The model under review builds one solid part; all positions refer to its coordinate system, in mm. Give positions to 0.01 mm unless a question says otherwise; leave off trailing zeros. Order: outer loops, then holes, each group sorted by start corner. A loop starts at its lowest first (then second) coordinate and runs counter-clockwise, first axis right, second up. Notation, with made-up numbers: M 70,16.5 L 87,16.5 A23 cw 87,49.5 Z; hole C -30.5,89 d3. An arc over 180 degrees is marked long. One line per question, with ' | ' between items. Start each with the question number.
1. Wall thickness on L1, parallel to X at y = 83.5, z = 4.25; L2, parallel to Y at x = -50.5, z = 9.5; L3, parallel to Y at x = -45, z = 12.5: over which ranges is each line inside the solid? List them lowest first.
2. We need section D-D on y = 108.5. Write out the cut boundary in (x, z).
3. We need section A-A on y = 63.5. Write out the cut boundary in (x, z).
4. Insertion check: P1, Ø1, axis at x = -27, y = 61.5, coming from the -Z side; P2, Ø10, axis at x = -10, z = 8, coming from the +Y side; P3, Ø10, axis at y = 93.5, z = 5, coming from the +X side; P4, Ø24, axis at x = -45, y = 81, coming from the -Z side. Each pin has a flat end and moves straight along its axis. Give the tip position at first contact, or say it passes through.
5. We need section B-B on x = -30. Write out the cut boundary in (y, z).
6. The part is to be moulded in two halves that separate along X. For faces 1 (the face through (-54.229, 63.257, 9.86)), 2 (the face through (-46, 50, 20)), 3 (the face through (-45.63, 6.785, 9.86)), say which applies: +X half, -X half, draft (parallel to the pull), parting line (faces both ways), or undercut.
7. We need section C-C on z = 4. Write out the cut boundary in (x, y).
```python
from build123d import *

# Parameters (mm, degrees)
EXTRUDE_1_DEPTH     = 20
SKETCH_2_R          = 20
CUT_EXTRUDE_1_DEPTH = 157.12815249


with BuildPart() as part:
    # 草图1 → 凸台-拉伸1 (new body)
    with BuildSketch(Plane.XY):
        with BuildLine():
            Line((0, 0), (0, 81))
            ThreePointArc((0, 81), (-45, 126), (-90, 81))
            Line((-90, 81), (-90, 13.383545734))
            Line((-90, 13.383545734), (0, 0))
        make_face()
    extrude(amount=EXTRUDE_1_DEPTH)

    # 草图2 → 切除-拉伸1 (cut, through all)
    with BuildSketch(Plane(origin=(0, 0, 0), x_dir=(-1, 0, 0), z_dir=(0, 0, -1))):
        with Locations((45, 81)):
            Circle(SKETCH_2_R)
    extrude(amount=-CUT_EXTRUDE_1_DEPTH, mode=Mode.SUBTRACT)


solid = part.part
```
Entries:
1) L1: x = -89.93 to -64.84, -25.16 to -0.07 | L2: y = 7.51 to 61.77, 100.23 to 125.66 | L3: y = 6.69 to 61, 101 to 126
2) outline: M -80.62,0 L -9.38,0 L -9.38,20 L -80.62,20 Z
3) outline: M -90,0 L -54.68,0 L -54.68,20 L -90,20 Z; M -35.32,0 L 0,0 L 0,20 L -35.32,20 Z
4) P1: stops at z = 0 | P2: stops at y = 114.54 | P3: stops at x = -0.63 | P4: passes through
5) outline: M 4.46,0 L 67.77,0 L 67.77,20 L 4.46,20 Z; M 94.23,0 L 123.43,0 L 123.43,20 L 94.23,20 Z
6) face 1: undercut | face 2: draft | face 3: -X half
7) outline: M -90,13.38 L 0,0 L 0,81 A45 ccw -90,81 Z; hole C -45,81 d40
